Part model, mm, in its own coordinate system. A direction names the side the tool comes from. Coordinates: 2 decimals unless noted, no trailing zeros. Loops run counter-clockwise (first coordinate to the right, second up) from the corner with the lowest first, then second, coordinate; pieces in that order, holes last. Notation, with made-up numbers: (72.5, 19.25) -> (91.5, 19.25) arc R15 cw to (91.5, 37.25) -> close; hole circle Ø3 at (47.25, 45). An arc over 180 degrees is marked (long way). One line per question, with ' | ' between items. Start each with the question number.
1) Cut at A-A (x = 0). List the corners of the cut face in (y, z).
2) Probe L1, parallel to Y at x = 0, z = 45.25; L2, parallel to Z at x = 13, y = 60; L3, parallel to X at y = 11.75, z = 100. List the from-to ranges inside material, lowest first. Write a range as from..to.
3) Cut at C-C (y = 66). List the corners of the cut face in (x, z).
4) Two-plate mould, pull along Y, no slides. Class faces 1 (the face through (-3.58, 177.266, 45.21)), 2 (the face through (-47.447, 89.28, -45.21)), 3 (the face through (40.979, 12.675, 131.445)): released by +Y, released by -Y, zero draft, split by the parting line, or undercut.
5) 3-axis set-ups, long thin cutter, end or side, ignore diameter. For faces 4 (the face through (-1, 92, -30)), 5 (the face through (0, 12, -140)), 6 (the face through (-1, 92, -60)): which of +Z, -Z, +X, -X, +Y, -Y reach the whole face in a straight line?
6) Cut at B-B (z = 100). List the corners of the cut face in (x, y).
7) Drop flat-ended pins along their axis: pin 1 (2 mm diameter, centred on x = -21.5, z = -106.5, fed in from +Y); pin 2 (2 mm diameter, centred on y = 156, z = 58, fed in from -X); pin 3 (12 mm diameter, centred on x = -23, y = 100, fed in from +Z). Give the stop position or say it passes through.
8) Cut at D-D (z = -44). List the corners of the cut face in (x, y), plus the area to 3 significant figures.
from build123d import *

# Parameters (mm, degrees)
SKETCH_1_W           = 100
SKETCH_1_H           = 120
BOSS_EXTRUDE_1_DEPTH = 25
SKETCH_2_R           = 27.5
BOSS_EXTRUDE_2_DEPTH = 30
SKETCH_4_W           = 15
SKETCH_4_H           = 25
BOSS_EXTRUDE_3_DEPTH = 10
SKETCH_5_W           = 100
SKETCH_5_H           = 280
SKETCH_5_R           = 13
BOSS_EXTRUDE_4_DEPTH = 25
FILLET_1_R           = 30


with BuildPart() as part:
    # Sketch 1 → Boss-Extrude 1 (new body)
    with BuildSketch(Plane(origin=(0, 0, 0), x_dir=(1, 0, 0), z_dir=(0, 1, 0))):
        Rectangle(SKETCH_1_W, SKETCH_1_H)
    extrude(amount=BOSS_EXTRUDE_1_DEPTH)

    # Sketch 2 → Boss-Extrude 2 (add)
    with BuildSketch(Plane.XY.offset(60)):
        with BuildLine():
            Line((-44.964550988, 151.785820395), (-50, 25))
            Line((-50, 25), (50, 25))
            Line((50, 25), (44.964550988, 151.785820395))
            ThreePointArc((44.964550988, 151.785820395), (0, 195), (-44.964550988, 151.785820395))
        make_face()
        with Locations((0, 150)):
            Circle(SKETCH_2_R, mode=Mode.SUBTRACT)
    boss_extrude_2 = extrude(amount=-BOSS_EXTRUDE_2_DEPTH)

    # Sketch 4 → Boss-Extrude 3 (add)
    with BuildSketch(Plane.XY.offset(60)):
        with Locations((0, 12.5)):
            Rectangle(SKETCH_4_W, SKETCH_4_H)
    boss_extrude_3 = extrude(amount=BOSS_EXTRUDE_3_DEPTH)

    # Mirror 1: Boss-Extrude 2, Boss-Extrude 3 across plane
    add(boss_extrude_2.mirror(Plane.XY))
    add(boss_extrude_3.mirror(Plane.XY))

    # Sketch 5 → Boss-Extrude 4 (add)
    with BuildSketch(Plane.XZ):
        Rectangle(SKETCH_5_W, SKETCH_5_H)
        with Locations(Location((0, -100, 0), (0, 0, 270))):
            Circle(SKETCH_5_R, mode=Mode.SUBTRACT)
        with Locations(Location((0, 100, 0), (0, 0, 270))):
            Circle(SKETCH_5_R, mode=Mode.SUBTRACT)
    extrude(amount=-BOSS_EXTRUDE_4_DEPTH)

    # Fillet 1
    fillet_1_edges = [part.edges().sort_by_distance(p)[0] for p in [
        (-50, 12.5, -140),
        (50, 12.5, 140),
        (50, 12.5, -140),
        (-50, 12.5, 140),
    ]]
    fillet(fillet_1_edges, radius=FILLET_1_R)


solid = part.part
Reported:
1) outline: (0, -140) -> (25, -140) -> (25, -113) -> (0, -113) -> close; (0, -87) -> (25, -87) -> (25, -60) -> (122.5, -60) -> (122.5, -30) -> (25, -30) -> (25, 30) -> (122.5, 30) -> (122.5, 60) -> (25, 60) -> (25, 87) -> (0, 87) -> close; (0, 113) -> (25, 113) -> (25, 140) -> (0, 140) -> close; (177.5, -60) -> (195, -60) -> (195, -30) -> (177.5, -30) -> close; (177.5, 30) -> (195, 30) -> (195, 60) -> (177.5, 60) -> close
2) L1: y = 0..122.5, 177.5..195 | L2: z = -60..-30, 30..60 | L3: x = -50..-13, 13..50
3) outline: (-48.37, -60) -> (48.37, -60) -> (48.37, -30) -> (-48.37, -30) -> close; (-48.37, 30) -> (48.37, 30) -> (48.37, 60) -> (-48.37, 60) -> close
4) face 1: undercut | face 2: released by +Y | face 3: zero draft
5) face 4: +X, -X, +Y | face 5: -Z, +X, -X, +Y, -Y | face 6: -Z, +X, -X, +Y
6) outline: (-50, 0) -> (-13, 0) -> (-13, 25) -> (-50, 25) -> close; (13, 0) -> (50, 0) -> (50, 25) -> (13, 25) -> close
7) pin 1: stops at y = 25 | pin 2: stops at x = -44.72 | pin 3: stops at z = 60
8) outline: (-50, 0) -> (50, 0) -> (50, 25) -> (44.96, 151.79) arc R45 ccw to (-44.96, 151.79) -> (-50, 25) -> close; hole circle Ø55 at (0, 150) | area: 15,200 mm²
